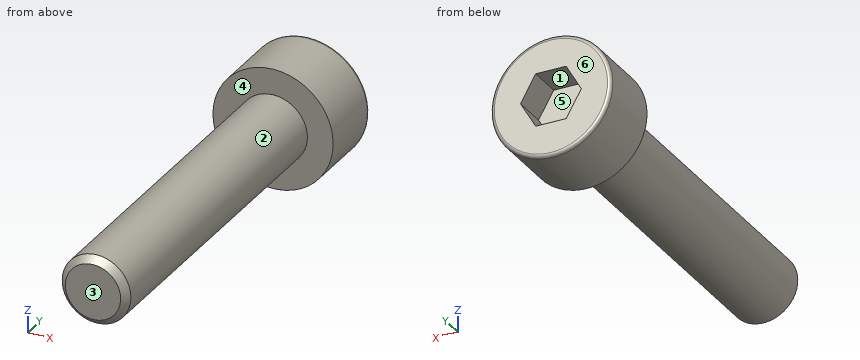
from build123d import *

# Parameters (mm, degrees)
SKETCH_1_R          = 3.5
EXTRUDE_1_DEPTH     = 4
CUT_EXTRUDE_1_DEPTH = 2
FILLET_1_R          = 0.2
SKETCH_5_R          = 2
EXTRUDE_2_DEPTH     = 20
CHAMFER_2_SIZE      = 0.39


with BuildPart() as part:
    # 草图1 → 凸台-拉伸1 (new body)
    with BuildSketch(Plane(origin=(0, 0, 0), x_dir=(1, 0, 0), z_dir=(0, 1, 0))):
        with Locations(Location((0, 0, 0), (0, 0, 270))):
            Circle(SKETCH_1_R)
    extrude(amount=EXTRUDE_1_DEPTH)

    # 草图2 → 切除-拉伸1 (cut)
    with BuildSketch(Plane(origin=(0, 4, 0), x_dir=(1, 0, 0), z_dir=(0, 1, 0))):
        Polygon((1.772465326, 0), (0.886232663, 1.535), (-0.886232663, 1.535), (-1.772465326, 0), (-0.886232663, -1.535), (0.886232663, -1.535), align=None)
    extrude(amount=-CUT_EXTRUDE_1_DEPTH, mode=Mode.SUBTRACT)

    # 圆角1
    fillet_1_edges = [part.edges().sort_by_distance(p)[0] for p in [
        (0, 4, -3.5),
    ]]
    fillet(fillet_1_edges, radius=FILLET_1_R)

    # 草图5 → 凸台-拉伸2 (add)
    with BuildSketch(Plane.XZ):
        with Locations(Location((0, 0, 0), (0, 0, 90))):
            Circle(SKETCH_5_R)
    extrude(amount=EXTRUDE_2_DEPTH)

    # 倒角2
    chamfer_2_edges = [part.edges().sort_by_distance(p)[0] for p in [
        (0, -20, -2),
    ]]
    chamfer(chamfer_2_edges, length=CHAMFER_2_SIZE)


solid = part.part
Check sheet for the modelled part. Datum: model origin and axes. Units: mm. Face numbers are marked on the shaded views. A direction names the side the tool comes from. Give positions to 0.01 mm unless a question says otherwise; leave off trailing zeros. Loops run counter-clockwise (first coordinate to the right, second up) from the corner with the lowest first, then second, coordinate; pieces in that order, holes last. Notation, with made-up numbers: M -4.5,54 L 49.5,54 A10 ccw 49.5,63 Z; hole C 0,72 d1. An arc over 180 degrees is marked long. Use a Markdown table: item, result. Add a question column.
Q1. Tool access check on the marked faces 4, 5 and 6. Record the directions out of +Z, -Z, +X, -X, +Y, -Y that give a thin tool (end or side, any length) a straight path to the whole face; none if there is none.
Q2. Sectioned sample at C-C, the plane y = -2. Record the cut outline in (x, z), then the cut area to 3 significant figures.
Q3. Scan lines: line 1 along Y through (x, z) = (0, -0.5); line 2 along Y through (x, z) = (-1.75, 2.75); line 3 along X through (y, z) = (-4, 0). Record each from-to range of solid material in increasing order. Write a range as [from, to].
Q4. Sectioned sample at A-A, the plane x = 0. Record the cut outline in (y, z) (3 decimals).
Q5. Go/stop test with flat-tipped pins: pin 1 (1.4 mm diameter, centred on x = -0.5, y = 3, fed in from -Z); pin 2 (1.5 mm diameter, centred on x = -0.5, z = -0.5, fed in from +Y). Record where each tip stops, or that it passes through.
Q6. Sectioned sample at B-B, the plane y = 1.25. Record the cut outline in (x, z).
Q7. Mould release check, pull along X, two halves, no side actions. Record for the marked faces 1, 2 and 3: pulls with the +X half, pulls with the -X half, needs draft (parallel to the pull), parting line crosses it, or undercut.
Verdict:
| question | item | result |
|---|---|---|
| 1 | face 4 | -Y |
| 1 | face 5 | +Y |
| 1 | face 6 | +Z, -Z, +X, -X, +Y |
| 2 | outline | C 0,0 d4 |
| 2 | area | 12.6 mm^2 |
| 3 | line 1 | [-20, 2] |
| 3 | line 2 | [0, 4] |
| 3 | line 3 | [-2, 2] |
| 4 | outline | M -20,-1.61 L -19.61,-2 L 0,-2 L 0,-3.5 L 3.8,-3.5 A0.2 ccw 4,-3.3 L 4,-1.535 L 2,-1.535 L 2,1.535 L 4,1.535 L 4,3.3 A0.2 ccw 3.8,3.5 L 0,3.5 L 0,2 L -19.61,2 L -20,1.61 Z |
| 5 | pin 1 | z = -3.5 |
| 5 | pin 2 | y = 2 |
| 6 | outline | C 0,0 d7 |
| 7 | face 1 | undercut |
| 7 | face 2 | parting line crosses it |
| 7 | face 3 | needs draft |
